Check sheet for the modelled part. Datum: model origin and axes. Units: mm. Face numbers are marked on the shaded views. A direction names the side the tool comes from. Coordinates: 2 decimals unless noted, no trailing zeros. Loops run counter-clockwise (first coordinate to the right, second up) from the corner with the lowest first, then second, coordinate; pieces in that order, holes last. Notation, with made-up numbers: (23.25, -5.75) -> (60.25, -5.75) arc R20 cw to (60.25, 8.25) -> close; hole circle Ø7 at (-15, 15.5). An arc over 180 degrees is marked (long way). Use CSV: the item, a comma, the result in double quotes.
```python
from build123d import *

# Parameters (mm, degrees)
MAIN_BODY_DEPTH                 = 65
CENTER_PAD_SKETCH_W             = 65
CENTER_PAD_SKETCH_H             = 28
CENTER_PAD_DEPTH                = 18
VERTICAL_BOSS_SKETCH_R          = 32.5
VERTICAL_BOSS_DEPTH             = 48
VERTICAL_START                  = 10
VERTICAL_BOSS_COLLAR_SKETCH_R   = 32.5
VERTICAL_BOSS_COLLAR_DEPTH      = 10
VERTICAL_START_2                = -10
VERTICAL_BOSS_RELIEF_SKETCH_R   = 32.5
VERTICAL_BOSS_RELIEF_CUT_DEPTH  = 10
VERTICAL_BORE_SKETCH_R          = 10
VERTICAL_BORE_20_DEPTH          = 48
ARM_DEPTH                       = 60
HORIZONTAL_BOSS_SKETCH_R        = 30
HORIZONTAL_BOSS_DEPTH           = 40
HORIZONTAL_START                = 10
HORIZONTAL_BOSS_COLLAR_SKETCH_R = 30
HORIZONTAL_BOSS_COLLAR_DEPTH    = 10
HORIZONTAL_BORE_SKETCH_R        = 12.5
HORIZONTAL_BORE_25_DEPTH        = 50


with BuildPart() as part:
    # Main Body Sketch → Main Body (new body)
    with BuildSketch(Plane.XY):
        Polygon((0, -28), (0, 0), (50, 0), (50, 32), (68, 32), (68, -28), align=None)
    extrude(amount=MAIN_BODY_DEPTH)

    # Center Pad Sketch → Center Pad (add)
    with BuildSketch(Plane.ZY):
        with Locations((32.5, -14)):
            Rectangle(CENTER_PAD_SKETCH_W, CENTER_PAD_SKETCH_H)
    extrude(amount=CENTER_PAD_DEPTH)

    # Vertical Boss Sketch → Vertical Boss (add)
    with BuildSketch(Plane(origin=(0, 0, 0), x_dir=(1, 0, 0), z_dir=(0, 1, 0))):
        with Locations(Location((-18, -32.5, 0), (0, 0, 270))):
            Circle(VERTICAL_BOSS_SKETCH_R)
    extrude(amount=-VERTICAL_BOSS_DEPTH)

    # Vertical Boss Collar Sketch → Vertical Boss Collar (add)
    with BuildSketch(Plane(origin=(0, 0, 0), x_dir=(1, 0, 0), z_dir=(0, 1, 0)).offset(VERTICAL_START)):
        with Locations(Location((-18, -32.5, 0), (0, 0, 270))):
            Circle(VERTICAL_BOSS_COLLAR_SKETCH_R)
    extrude(amount=-VERTICAL_BOSS_COLLAR_DEPTH)

    # Vertical Boss Relief Sketch → Vertical Boss Relief Cut (cut)
    with BuildSketch(Plane.XZ.offset(48).offset(VERTICAL_START_2)):
        with Locations(Location((-18, 32.5, 0), (0, 0, 90))):
            Circle(VERTICAL_BOSS_RELIEF_SKETCH_R)
    extrude(amount=VERTICAL_BOSS_RELIEF_CUT_DEPTH, mode=Mode.SUBTRACT)

    # Vertical Bore Sketch → Vertical Bore Ø20 (cut)
    with BuildSketch(Plane(origin=(0, 10, 0), x_dir=(1, 0, 0), z_dir=(0, 1, 0))):
        with Locations(Location((-18, -32.5, 0), (0, 0, 270))):
            Circle(VERTICAL_BORE_SKETCH_R)
    extrude(amount=-VERTICAL_BORE_20_DEPTH, mode=Mode.SUBTRACT)

    # Arm Sketch → Arm (add)
    with BuildSketch(Plane(origin=(0, 32, 0), x_dir=(1, 0, 0), z_dir=(0, 1, 0))):
        Polygon((140, -32.5), (140, -17.5), (68, -17.5), (68, -47.5), (140, -47.5), align=None)
    extrude(amount=-ARM_DEPTH)

    # Horizontal Boss Sketch → Horizontal Boss (add)
    with BuildSketch(Plane.XY.offset(47.5)):
        with Locations((140, 2)):
            Circle(HORIZONTAL_BOSS_SKETCH_R)
    extrude(amount=-HORIZONTAL_BOSS_DEPTH)

    # Horizontal Boss Collar Sketch → Horizontal Boss Collar (add)
    with BuildSketch(Plane.XY.offset(47.5).offset(HORIZONTAL_START)):
        with Locations((140, 2)):
            Circle(HORIZONTAL_BOSS_COLLAR_SKETCH_R)
    extrude(amount=-HORIZONTAL_BOSS_COLLAR_DEPTH)

    # Horizontal Bore Sketch → Horizontal Bore Ø25 (cut)
    with BuildSketch(Plane.XY.offset(57.5)):
        with Locations((140, 2)):
            Circle(HORIZONTAL_BORE_SKETCH_R)
    extrude(amount=-HORIZONTAL_BORE_25_DEPTH, mode=Mode.SUBTRACT)


solid = part.part
```
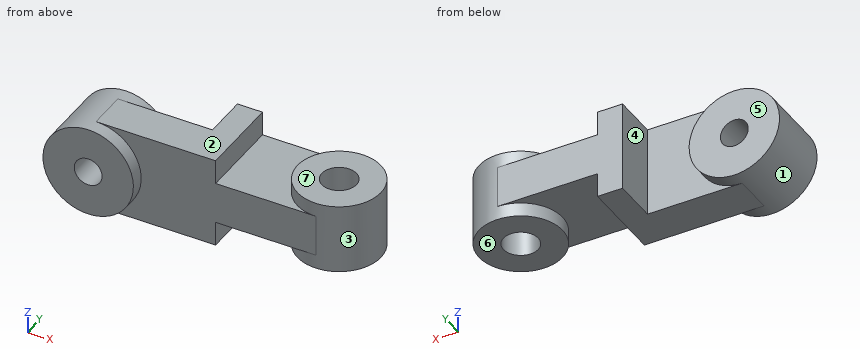
1) Go/stop test with flat-tipped pins: pin 1 Ø19.5 at (x, z) = (-9.5, 21) entering from +Y; pin 2 Ø5 at (y, z) = (14, 10.5) entering from -X; pin 3 Ø10 at (x, y) = (118, 12) entering from -Z. Record where each tip stops, or that it passes through.
Answer below:
pin 1,"stops at y = 10"
pin 2,"stops at x = 50"
pin 3,"stops at z = 7.5"
2) Thickness scan on line 1 along Y through (x, z) = (140, 21); line 2 along X through (y, z) = (-9.5, 50.5); line 3 along X through (y, z) = (-7, 34). Record the ranges inside material, lowest first. Write a range as from..to.
Answer below:
line 1,"y = -28..-10.5, 14.5..32"
line 2,"x = -45.06..68, 112.29..135.1, 144.9..167.71"
line 3,"x = -50.47..-27.89, -8.11..131.33, 148.67..168.62"
3) Cross-section at C-C on x = 145. Record the boundary of the cut face in (y, z).
Answer below:
outline,"(-27.58, 7.5) -> (-9.46, 7.5) -> (-9.46, 57.5) -> (-27.58, 57.5) -> close; (13.46, 7.5) -> (31.58, 7.5) -> (31.58, 57.5) -> (13.46, 57.5) -> close"
4) Cross-section at D-D on z = 11. Record the boundary of the cut face in (x, y), and give its area (3 significant figures).
Answer below:
outline,"(-42.37, -38) -> (6.37, -38) -> (6.37, -28) -> (68, -28) -> (68, 32) -> (50, 32) -> (50, 0) -> (6.37, 0) -> (6.37, 10) -> (-42.37, 10) -> close; circle Ø60 at (140, 2); hole circle Ø25 at (140, 2)"
area,"6,980 mm²"
5) Draft check along X on the marked faces 1 and 2. Enter one of: released by +X, released by -X, zero draft, split by the parting line, or undercut.
Answer below:
face 1,"undercut"
face 2,"zero draft"
6) Cross-section at B-B on y = -13. Record the boundary of the cut face in (x, z).
Answer below:
outline,"(-18, 0) -> (68, 0) -> (68, 17.5) -> (114.02, 17.5) -> (114.02, 7.5) -> (165.98, 7.5) -> (165.98, 57.5) -> (114.02, 57.5) -> (114.02, 47.5) -> (68, 47.5) -> (68, 65) -> (-18, 65) arc R32.5 ccw to start; hole circle Ø20 at (-18, 32.5)"
7) Access from +Z, -Z, +X, -X, +Y, -Y to the whole of each face (thin tool, end or side, straight path). Record for the marked faces 3, 4, 5, 6 and 7.
Answer below:
face 3,"none"
face 4,"+Z, -Z, +Y"
face 5,"+Z, -Z, -X, +Y"
face 6,"-Z, +X, +Y, -Y"
face 7,"+Z, +X, +Y, -Y"
8) Cross-section at A-A on z = 32.5. Record the boundary of the cut face in (x, y), and give its area (3 significant figures).
Answer below:
outline,"(-50.5, -38) -> (-28, -38) -> (-28, 10) -> (-50.5, 10) -> close; (-8, -38) -> (14.5, -38) -> (14.5, -28) -> (140, -28) arc R30 ccw to (140, 32) -> (50, 32) -> (50, 0) -> (14.5, 0) -> (14.5, 10) -> (-8, 10) -> close; hole circle Ø25 at (140, 2)"
area,"9,480 mm²"
